Check sheet for the drawn part. Datum: minimum x, y, z corner. Units: mm. Coordinates: 2 decimals unless noted, no trailing zeros. Write each loop counter-clockwise with the first axis right and the second up, starting at its lowest first coordinate (ties: lowest second). Pieces come first, ordered by that corner, then holes. Notation, with made-up numbers: (70.5, 27) - (119.5, 27) arc R17 cw to (119.5, 39) - close; hole circle Ø3 at (49.5, 36). An arc over 180 degrees is marked (long way). Use one line per item in the form item = value. Start each with the question number.
1. Draft check along Y on the marked faces 1, 2 and 3. Enter one of: +Y half, -Y half, draft (parallel to the pull), parting line (faces both ways), or undercut.
2. Cross-section at C-C on x = 85. Record the boundary of the cut face in (y, z), then the cut area to 3 significant figures.
3. Cross-section at A-A on y = 70. Record the boundary of the cut face in (x, z), then the cut area to 3 significant figures.
4. Scan lines: line 1 along Y through (x, z) = (85, 6); line 2 along Y through (x, z) = (10, 3.25); line 3 along X through (y, z) = (9, 9.25). Record each from-to range of solid material in increasing order.
5. Go/stop test with a flat-tipped pin: pin 1 Ø9 at (x, y) = (15, 10) entering from -Z. Record where the tip stops, or that it passes through.
6. Cross-section at B-B on z = 7.5. Record the boundary of the cut face in (x, y).
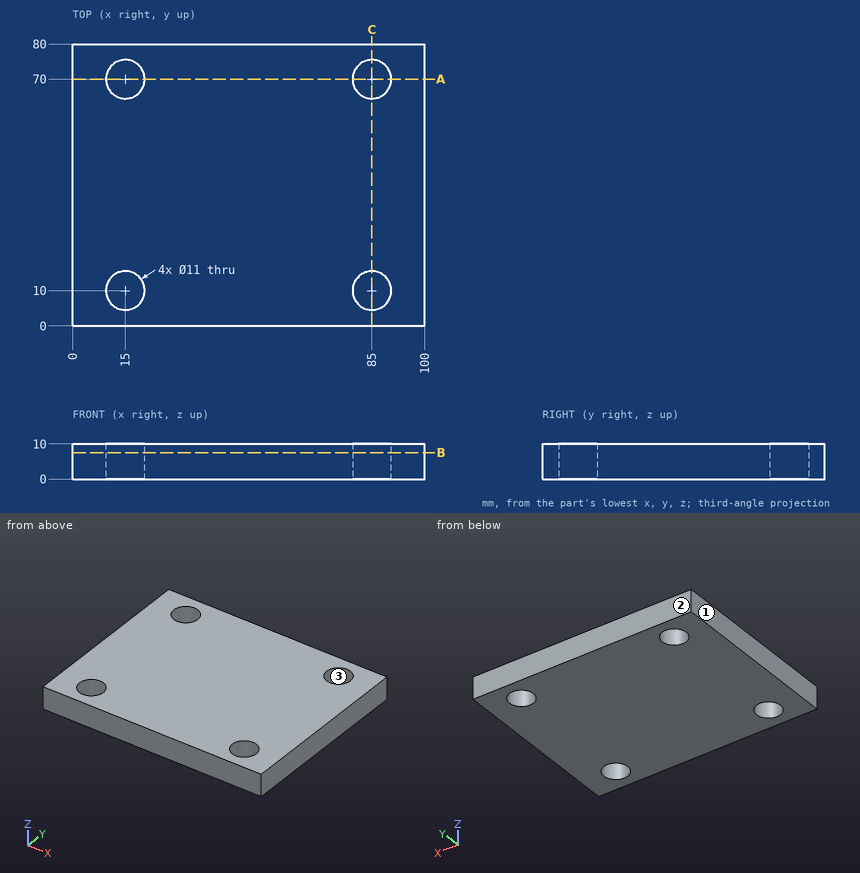
Final values:
q1.face_1 = draft
q1.face_2 = +Y half
q1.face_3 = undercut
q2.outline = (0, 0) - (4.5, 0) - (4.5, 10) - (0, 10) - close; (15.5, 0) - (64.5, 0) - (64.5, 10) - (15.5, 10) - close; (75.5, 0) - (80, 0) - (80, 10) - (75.5, 10) - close
q2.area = 580 mm²
q3.outline = (0, 0) - (9.5, 0) - (9.5, 10) - (0, 10) - close; (20.5, 0) - (79.5, 0) - (79.5, 10) - (20.5, 10) - close; (90.5, 0) - (100, 0) - (100, 10) - (90.5, 10) - close
q3.area = 780 mm²
q4.line_1 = 0 to 4.5, 15.5 to 64.5, 75.5 to 80
q4.line_2 = 0 to 7.71, 12.29 to 67.71, 72.29 to 80
q4.line_3 = 0 to 9.59, 20.41 to 79.59, 90.41 to 100
q5.pin_1 = through
q6.outline = (0, 0) - (100, 0) - (100, 80) - (0, 80) - close; hole circle Ø11 at (15, 10); hole circle Ø11 at (15, 70); hole circle Ø11 at (85, 10); hole circle Ø11 at (85, 70)
